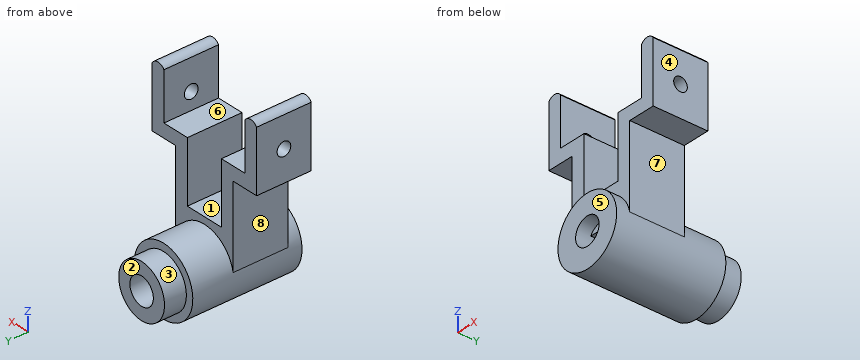
from build123d import *

# Parameters (mm, degrees)
MAIN_BOSS_SKETCH_50_R  = 25
MAIN_BOSS_50X80_DEPTH  = 80
TOP_STEP_SKETCH_39_R   = 19.5
TOP_STEP_39X16_DEPTH   = 16
BORE_SKETCH_20_R       = 10
BORE_20_DEPTH          = 103.303470127
BRACKET_BLOCK_SKETCH_W = 49
BRACKET_BLOCK_SKETCH_H = 60
BRACKET_BLOCK_DEPTH    = 40
BRACKET_SLOT_SKETCH_W  = 29
BRACKET_SLOT_SKETCH_H  = 35
BRACKET_SLOT_DEPTH     = 40
MOUNTING_LUGS_DEPTH    = 40
LUG_HOLE_SKETCH_10_R   = 5
LUG_HOLES_10_DEPTH     = 173.710437877


with BuildPart() as part:
    # Main Boss Sketch Ø50 → Main Boss Ø50x80 (new body)
    with BuildSketch(Plane(origin=(0, 0, 0), x_dir=(1, 0, 0), z_dir=(0, 1, 0))):
        with Locations(Location((0, 0, 0), (0, 0, 270))):
            Circle(MAIN_BOSS_SKETCH_50_R)
    extrude(amount=MAIN_BOSS_50X80_DEPTH)

    # Top Step Sketch Ø39 → Top Step Ø39x16 (add)
    with BuildSketch(Plane(origin=(0, 80, 0), x_dir=(1, 0, 0), z_dir=(0, 1, 0))):
        with Locations(Location((0, 0, 0), (0, 0, 270))):
            Circle(TOP_STEP_SKETCH_39_R)
    extrude(amount=TOP_STEP_39X16_DEPTH)

    # Bore Sketch Ø20 → Bore Ø20 (cut, through all)
    with BuildSketch(Plane(origin=(0, 96, 0), x_dir=(1, 0, 0), z_dir=(0, 1, 0))):
        with Locations(Location((0, 0, 0), (0, 0, 270))):
            Circle(BORE_SKETCH_20_R)
    extrude(amount=-BORE_20_DEPTH, mode=Mode.SUBTRACT)

    # Bracket Block Sketch → Bracket Block (add)
    with BuildSketch(Plane(origin=(0, 10, 0), x_dir=(1, 0, 0), z_dir=(0, 1, 0))):
        with Locations((0, -34.974937186)):
            Rectangle(BRACKET_BLOCK_SKETCH_W, BRACKET_BLOCK_SKETCH_H)
    extrude(amount=BRACKET_BLOCK_DEPTH)

    # Bracket Slot Sketch → Bracket Slot (cut)
    with BuildSketch(Plane(origin=(0, 50, 0), x_dir=(1, 0, 0), z_dir=(0, 1, 0))):
        with Locations((0, -47.474937186)):
            Rectangle(BRACKET_SLOT_SKETCH_W, BRACKET_SLOT_SKETCH_H)
    extrude(amount=-BRACKET_SLOT_DEPTH, mode=Mode.SUBTRACT)

    # Mounting Lugs Sketch → Mounting Lugs (add)
    with BuildSketch(Plane(origin=(0, 50, 0), x_dir=(1, 0, 0), z_dir=(0, 1, 0))):
        with BuildLine():
            Line((14.5, -64.974937186), (44.5, -64.974937186))
            Line((44.5, -64.974937186), (44.5, -74.974937186))
            Line((44.5, -74.974937186), (44.5, -109.974937186))
            ThreePointArc((44.5, -109.974937186), (39.5, -112.658312395), (34.5, -109.974937186))
            Line((34.5, -109.974937186), (34.5, -74.974937186))
            Line((34.5, -74.974937186), (14.5, -74.974937186))
            Line((14.5, -74.974937186), (14.5, -64.974937186))
        make_face()
        with BuildLine():
            Line((-14.5, -64.974937186), (-44.5, -64.974937186))
            Line((-44.5, -64.974937186), (-44.5, -74.974937186))
            Line((-44.5, -74.974937186), (-44.5, -109.974937186))
            ThreePointArc((-44.5, -109.974937186), (-39.5, -112.658312395), (-34.5, -109.974937186))
            Line((-34.5, -109.974937186), (-34.5, -74.974937186))
            Line((-34.5, -74.974937186), (-14.5, -74.974937186))
            Line((-14.5, -74.974937186), (-14.5, -64.974937186))
        make_face()
    extrude(amount=-MOUNTING_LUGS_DEPTH)

    # Lug Hole Sketch Ø10 → Lug Holes Ø10 (cut, through all)
    with BuildSketch(Plane(origin=(44.5, 0, 0), x_dir=(0, 0, -1), z_dir=(1, 0, 0))):
        with Locations((-87.474937186, 30)):
            Circle(LUG_HOLE_SKETCH_10_R)
    extrude(amount=-LUG_HOLES_10_DEPTH, mode=Mode.SUBTRACT)


solid = part.part
Check sheet for the modelled part. Datum: model origin and axes. Units: mm. Face numbers are marked on the shaded views. A direction names the side the tool comes from. Coordinates: 2 decimals unless noted, no trailing zeros. Loops run counter-clockwise (first coordinate to the right, second up) from the corner with the lowest first, then second, coordinate; pieces in that order, holes last. Notation, with made-up numbers: (87.5, 61) -> (97.5, 61) arc R24 ccw to (97.5, 86) -> close; hole circle Ø6 at (57, 78). An arc over 180 degrees is marked (long way). Write item = value, one per line. Start each with the question number.
1. Section check A-A on y = 30. Record the cut outline in (x, z), then the cut area to 3 significant figures.
2. Depth check by flat-ended pin: P1, Ø4, axis at x = 27.5, z = 11.5, coming from the -Y side; P2, Ø20, axis at y = 34, z = 32.5, coming from the +X side; P3, Ø8.5, axis at x = 5.5, y = 27.5, coming from the +Z side; P4, Ø3, axis at x = 11, y = 33, coming from the -Z side. Enter the tip coordinate at first touch or a pass-through.
3. Material ranges on line 1 (X direction, y = 61.5, z = 0); line 2 (Y direction, x = 13, z = 16); line 3 (Y direction, x = -39, z = 89.5), recorded low to high.
4. Section check C-C on z = 0. Record the cut outline in (x, y).
5. Section check B-B on x = 0. Record the cut outline in (y, z).
6. Tool access check on the marked faces 4, 5, 6, 7 and 8. Record the directions out of +Z, -Z, +X, -X, +Y, -Y that give a thin tool (end or side, any length) a straight path to the whole face; none if there is none.
7. Section check D-D on z = 96. Record the cut outline in (x, y).
8. Draft check along X on the marked faces 1, 2 and 3. Enter one of: released by +X, released by -X, zero draft, split by the parting line, or undercut.
Responses:
q1.outline = (-44.5, 64.97) -> (-24.5, 64.97) -> (-24.5, 4.97) arc R25 ccw (long way) to (24.5, 4.97) -> (24.5, 64.97) -> (44.5, 64.97) -> (44.5, 82.47) -> (34.5, 82.47) -> (34.5, 74.97) -> (14.5, 74.97) -> (14.5, 29.97) -> (-14.5, 29.97) -> (-14.5, 74.97) -> (-34.5, 74.97) -> (-34.5, 82.47) -> (-44.5, 82.47) -> close; (-44.5, 92.47) -> (-34.5, 92.47) -> (-34.5, 109.97) arc R6 ccw to (-44.5, 109.97) -> close; (34.5, 92.47) -> (44.5, 92.47) -> (44.5, 109.97) arc R6 ccw to (34.5, 109.97) -> close; hole (-8.67, 4.97) arc R10 ccw (long way) to (8.67, 4.97) -> close
q1.area = 4,040 mm2
q2.P1 = through
q2.P2 = 24.5
q2.P3 = 29.97
q2.P4 = -23.12
q3.line_1 = -25 to -10, 10 to 25
q3.line_2 = 0 to 80
q3.line_3 = 10 to 25.43, 34.57 to 50
q4.outline = (-25, 0) -> (-10, 0) -> (-10, 96) -> (-19.5, 96) -> (-19.5, 80) -> (-25, 80) -> close; (10, 0) -> (25, 0) -> (25, 80) -> (19.5, 80) -> (19.5, 96) -> (10, 96) -> close
q5.outline = (0, -25) -> (80, -25) -> (80, -19.5) -> (96, -19.5) -> (96, -10) -> (0, -10) -> close; (0, 10) -> (10, 10) -> (10, 4.97) -> (50, 4.97) -> (50, 10) -> (96, 10) -> (96, 19.5) -> (80, 19.5) -> (80, 25) -> (50, 25) -> (50, 29.97) -> (10, 29.97) -> (10, 25) -> (0, 25) -> close
q6.face_4 = +Z, -Z, +X, +Y, -Y
q6.face_5 = +Z, -Z, +X, -X, -Y
q6.face_6 = +Z, +Y, -Y
q6.face_7 = +X, +Y, -Y
q6.face_8 = -X, +Y, -Y
q7.outline = (-44.5, 10) -> (-34.5, 10) -> (-34.5, 50) -> (-44.5, 50) -> close; (34.5, 10) -> (44.5, 10) -> (44.5, 50) -> (34.5, 50) -> close
q8.face_1 = undercut
q8.face_2 = zero draft
q8.face_3 = split by the parting line
